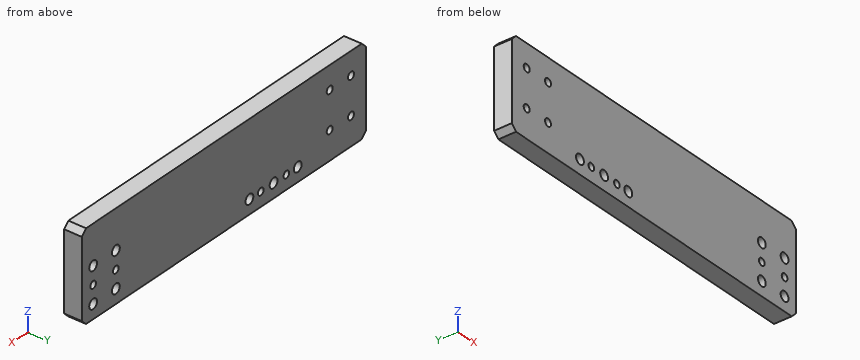
```python
from build123d import *

# Parameters (mm, degrees)
SKETCH_6_W                  = 200
SKETCH_6_H                  = 50
EXTRUDE_1_DEPTH             = 10
CHAMFER_1_SIZE              = 3
HOLE_WIZARD_5_5_5_5_1_D     = 5.5
HOLE_WIZARD_5_5_5_5_1_DEPTH = 12.4
HOLE_WIZARD_5_5_5_5_1_TIP   = 1.652366702
MM_2_D                      = 4
MM_2_DEPTH                  = 12.4
MM_2_TIP                    = 1.201721238
HOLE_WIZARD_M5_2_D          = 4.2
HOLE_WIZARD_M5_2_DEPTH      = 12.4
HOLE_WIZARD_M5_2_TIP        = 1.2618073
HOLE_WIZARD_5_5_5_5_2_D     = 5.5
HOLE_WIZARD_5_5_5_5_2_DEPTH = 12.4
HOLE_WIZARD_5_5_5_5_2_TIP   = 1.652366702
MM_3_D                      = 4
MM_3_DEPTH                  = 12.4
MM_3_TIP                    = 1.201721238


with BuildPart() as part:
    # 草图6 → 凸台-拉伸1 (new body)
    with BuildSketch(Plane(origin=(0, 0, 0), x_dir=(1, 0, 0), z_dir=(0, 1, 0))):
        Rectangle(SKETCH_6_W, SKETCH_6_H)
    extrude(amount=EXTRUDE_1_DEPTH)

    # 倒角1
    chamfer_1_edges = [part.edges().sort_by_distance(p)[0] for p in [
        (100, 5, 25),
        (-100, 5, 25),
        (-100, 5, -25),
        (100, 5, -25),
    ]]
    chamfer(chamfer_1_edges, length=CHAMFER_1_SIZE)

    # Ø5.5 (5.5) 直径孔1
    with Locations(Plane(origin=(0, 10, 0), x_dir=(1, 0, 0), z_dir=(0, 1, 0))):
        with Locations((76, 17), (76, -3), (92, -3), (92, 17)):
            Hole(HOLE_WIZARD_5_5_5_5_1_D / 2, depth=HOLE_WIZARD_5_5_5_5_1_DEPTH)
            with Locations((0, 0, -(HOLE_WIZARD_5_5_5_5_1_DEPTH + HOLE_WIZARD_5_5_5_5_1_TIP / 2))):  # 118° drill point
                Cone(0, HOLE_WIZARD_5_5_5_5_1_D / 2, HOLE_WIZARD_5_5_5_5_1_TIP, mode=Mode.SUBTRACT)

    # 大小mm 暗销孔2
    with Locations(Plane(origin=(0, 10, 0), x_dir=(1, 0, 0), z_dir=(0, 1, 0))):
        with Locations((76, 7), (92, 7)):
            Hole(MM_2_D / 2, depth=MM_2_DEPTH)
            with Locations((0, 0, -(MM_2_DEPTH + MM_2_TIP / 2))):  # 118° drill point
                Cone(0, MM_2_D / 2, MM_2_TIP, mode=Mode.SUBTRACT)

    # M5 螺纹孔2
    with Locations(Plane(origin=(0, 10, 0), x_dir=(1, 0, 0), z_dir=(0, 1, 0))):
        with Locations((-89.5, 9), (-74.5, 9), (-89.5, -12), (-74.5, -12)):
            Hole(HOLE_WIZARD_M5_2_D / 2, depth=HOLE_WIZARD_M5_2_DEPTH)
            with Locations((0, 0, -(HOLE_WIZARD_M5_2_DEPTH + HOLE_WIZARD_M5_2_TIP / 2))):  # 118° drill point
                Cone(0, HOLE_WIZARD_M5_2_D / 2, HOLE_WIZARD_M5_2_TIP, mode=Mode.SUBTRACT)

    # Ø5.5 (5.5) 直径孔2
    with Locations(Plane(origin=(0, 0, 0), x_dir=(-1, 0, 0), z_dir=(0, -1, 0))):
        with Locations((52, 17), (35, 16.974257895), (18, 16.974257895)):
            Hole(HOLE_WIZARD_5_5_5_5_2_D / 2, depth=HOLE_WIZARD_5_5_5_5_2_DEPTH)
            with Locations((0, 0, -(HOLE_WIZARD_5_5_5_5_2_DEPTH + HOLE_WIZARD_5_5_5_5_2_TIP / 2))):  # 118° drill point
                Cone(0, HOLE_WIZARD_5_5_5_5_2_D / 2, HOLE_WIZARD_5_5_5_5_2_TIP, mode=Mode.SUBTRACT)

    # 大小mm 暗销孔3
    with Locations(Plane(origin=(0, 0, 0), x_dir=(-1, 0, 0), z_dir=(0, -1, 0))):
        with Locations((44, 17), (26, 17)):
            Hole(MM_3_D / 2, depth=MM_3_DEPTH)
            with Locations((0, 0, -(MM_3_DEPTH + MM_3_TIP / 2))):  # 118° drill point
                Cone(0, MM_3_D / 2, MM_3_TIP, mode=Mode.SUBTRACT)


solid = part.part
```
Geometry check sheet. Reference: the model listing, model coordinates, mm. Round coordinates to 2 decimals unless told otherwise and drop trailing zeros. Loops run counter-clockwise (first coordinate to the right, second up) from the corner with the lowest first, then second, coordinate; pieces in that order, holes last. Notation, with made-up numbers: (35, 61.25) - (83, 61.25) arc R34 ccw to (83, 99.25) - close; hole circle Ø9 at (-15, 77). An arc over 180 degrees is marked (long way). Write item = value, one per line. Start each with the question number.
1. Section check A-A on z = 12. Enter the section's corners in (x, y), then the cut area to 3 significant figures.
2. Section check B-B on x = -89.5. Enter the section's corners in (y, z), then the cut area to 3 significant figures.
3. Thickness scan on line 1 (Z direction, x = 76, y = 5.25); line 2 (Z direction, x = -89.5, y = 5.75); line 3 (Z direction, x = -44, y = 3.75). Record the ranges inside material, lowest first.
4. Section check D-D on y = 5.5. Give the number of separate pieces and of enclosed holes in the cut face, then the cut area to 3 significant figures.
5. Depth check by flat-ended pin: pin 1 (4 mm diameter, centred on x = -89.5, z = 12, fed in from -Y). Enter the tip coordinate at first touch or a pass-through.
6. Section check C-C on x = -35. Enter the section's corners in (y, z), then the cut area to 3 significant figures.
Working result:
q1.outline = (-100, 0) - (-91.6, 0) - (-91.6, 10) - (-100, 10) - close; (-87.4, 0) - (-76.6, 0) - (-76.6, 10) - (-87.4, 10) - close; (-72.4, 0) - (100, 0) - (100, 10) - (-72.4, 10) - close
q1.area = 1,920 mm^2
q2.outline = (0, -25) - (10, -25) - (10, -11.1) - (0, -11.1) - close; (0, -6.9) - (10, -6.9) - (10, 9.9) - (0, 9.9) - close; (0, 14.1) - (10, 14.1) - (10, 25) - (0, 25) - close
q2.area = 416 mm^2
q3.line_1 = -25 to -19.75, -14.25 to -9, -5 to 0.25, 5.75 to 25
q3.line_2 = -25 to -11.1, -6.9 to 9.9, 14.1 to 25
q3.line_3 = -25 to -19, -15 to 25
q4.separate_pieces = 1
q4.enclosed_holes = 15
q4.area = 9,710 mm^2
q5.pin_1 = through
q6.outline = (0, -25) - (10, -25) - (10, -19.72) - (0, -19.72) - close; (0, -14.22) - (10, -14.22) - (10, 25) - (0, 25) - close
q6.area = 445 mm^2
